from build123d import *

# Parameters (mm, degrees)
SKETCH1_R           = 6
BOSS_EXTRUDE1_DEPTH = 10
BOSS_EXTRUDE2_DEPTH = 5
SKETCH3_R           = 6.018032789
BOSS_EXTRUDE3_DEPTH = 1
FILLET2_R           = 0.5


with BuildPart() as part:
    # Sketch1 → Boss-Extrude1 (new body)
    with BuildSketch(Plane.XY):
        Circle(SKETCH1_R)
    extrude(amount=BOSS_EXTRUDE1_DEPTH)

    # Sketch2 → Boss-Extrude2 (add)
    with BuildSketch(Plane.XY.offset(10)):
        Polygon((0, 7.285798141), (-6.309686277, 3.64289907), (-6.309686277, -3.64289907), (0, -7.285798141), (6.309686277, -3.64289907), (6.309686277, 3.64289907), align=None)
    extrude(amount=BOSS_EXTRUDE2_DEPTH)

    # Sketch3 → Boss-Extrude3 (add)
    with BuildSketch(Plane.XY.offset(15)):
        Circle(SKETCH3_R)
    extrude(amount=BOSS_EXTRUDE3_DEPTH)

    # Fillet2
    fillet2_edges = [part.edges().sort_by_distance(p)[0] for p in [
        (-6.018032789, 0, 16),
    ]]
    fillet(fillet2_edges, radius=FILLET2_R)


solid = part.part
Here's how the part is built. I have some questions about the finished solid (model axes, mm). A direction names the side the tool comes from. Coordinates: 2 decimals unless noted, no trailing zeros. Order: outer loops, then holes, each group sorted by start corner. A loop starts at its lowest first (then second) coordinate and runs counter-clockwise, first axis right, second up. Notation, with made-up numbers: M 44.5,21.25 L 59.5,21.25 A28 ccw 59.5,50.25 Z; hole C 67,70 d8. An arc over 180 degrees is marked long. Answer as CSV lines item,"result". Start each with the question number.
1. On a 3-axis mill with a long thin cutter (end or side, diameter ignored), from which of +Z, -Z, +X, -X, +Y, -Y can I reach the whole of each face in a straight line? I mean faces 1 (the cylindrical face through (-6, 0, 5)), 2 (the flat face through (-3.11, 5.49, 12.46)), 3 (the cylindrical face through (5.56, -2.3, 15.25)). Say none if no direction works.
2. I want a section at C-C, the plane z = 4.75. Write out the boundary of the cut face in (x, y).
3. For pin 1 (1 mm diameter, centred on y = -5.5, z = 11, fed in from +X); pin 2 (1 mm diameter, centred on y = 3, z = 8, fed in from +X), each with a flat end and sliding along its axis, tell me the tip position at first contact or that it passes through.
4. I want a section at B-B, the plane z = 13.25. Write out the boundary of the cut face in (x, y).
5. I want a section at A-A, the plane y = 0. Write out the boundary of the cut face in (x, z), and give its area (3 significant figures).
6. I need wall thicknesses on line 1 (Z direction, x = 0.5, y = 6.75); line 2 (X direction, y = 3.75, z = 2.5); line 3 (X direction, y = 3.5, z = 5.75). Which ranges of each line are inside material? Lowest first, please. Write a range as [from, to].
Recorded:
1,face 1,"-Z"
1,face 2,"+Z, -Z, -X, +Y"
1,face 3,"+Z"
2,outline,"C 0,0 d12"
3,pin 1,"stops at x = 3.96"
3,pin 2,"stops at x = 5.45"
4,outline,"M -6.31,-3.64 L 0,-7.29 L 6.31,-3.64 L 6.31,3.64 L 0,7.29 L -6.31,3.64 Z"
5,outline,"M -6.31,10 L -6,10 L -6,0 L 6,0 L 6,10 L 6.31,10 L 6.31,15 L 6.02,15 L 6.02,15.5 A0.5 ccw 5.52,16 L -5.52,16 A0.5 ccw -6.02,15.5 L -6.02,15 L -6.31,15 Z"
5,area,"195 mm2"
6,line 1,"z = [10, 15]"
6,line 2,"x = [-4.68, 4.68]"
6,line 3,"x = [-4.87, 4.87]"
